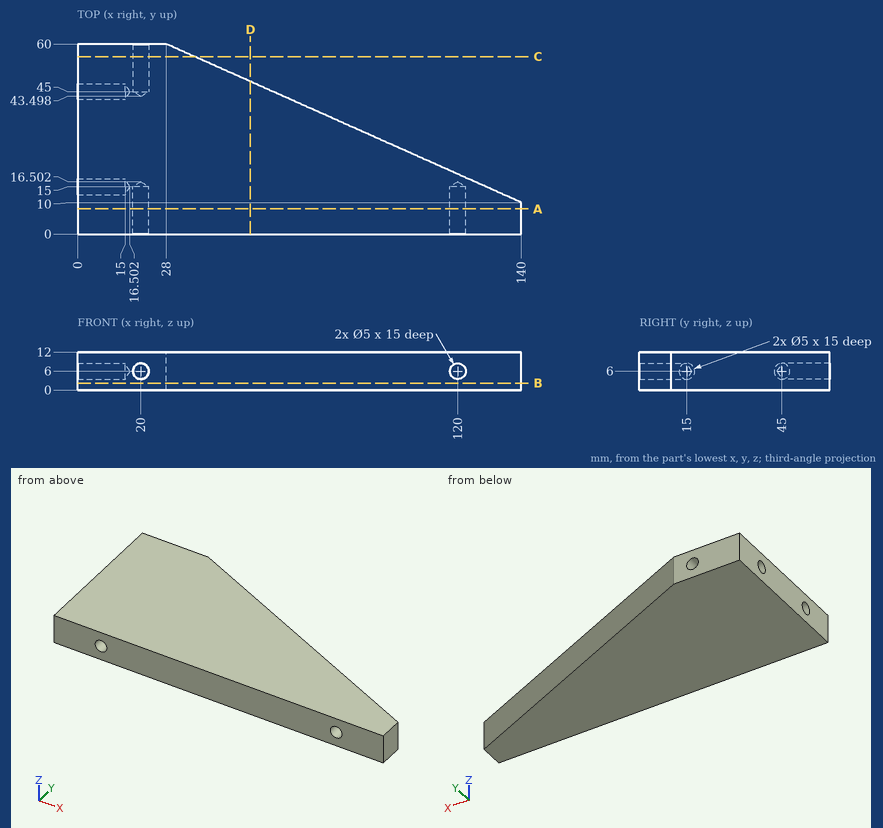
Part print with two shaded views. Sizes in mm from the minimum x, y, z corner. Round coordinates to 2 decimals unless told otherwise and drop trailing zeros. Order: outer loops, then holes, each group sorted by start corner. A loop starts at its lowest first (then second) coordinate and runs counter-clockwise, first axis right, second up. Notation, with made-up numbers: (14.25, -21.5) - (57.25, -21.5) arc R19 ccw to (57.25, -6.5) - close; hole circle Ø10 at (16, -27.5). An arc over 180 degrees is marked (long way). Answer in a Markdown table with one row per item. Add a question column.
(1) Band-saw the part on A-A on y = 8. List the corners of the cut face in (x, z).
(2) Band-saw the part on C-C on y = 56. List the corners of the cut face in (x, z).
(3) Band-saw the part on B-B on z = 2.25. List the corners of the cut face in (x, y).
(4) Probe L1, parallel to Y at x = 3.75, z = 6; L2, parallel to Z at x = 120, y = 8.25; L3, parallel to Y at x = 125.5, z = 11.5. List the from-to ranges inside material, lowest first. Write a range as [from, to].
(5) Band-saw the part on D-D on x = 54.5. List the corners of the cut face in (y, z).
(6) Drop flat-ended pins along their axis: pin 1 Ø3 at (x, z) = (20, 6) entering from +Y; pin 2 Ø5 at (x, z) = (122, 9) entering from +Y; pin 3 Ø4 at (y, z) = (45, 6) entering from +X. Give the stop position or say it passes through.
Data:
| question | item | result |
|---|---|---|
| 1 | outline | (0, 0) - (140, 0) - (140, 12) - (0, 12) - close; hole circle Ø5 at (20, 6); hole circle Ø5 at (120, 6) |
| 2 | outline | (0, 0) - (36.96, 0) - (36.96, 12) - (0, 12) - close; hole circle Ø5 at (20, 6) |
| 3 | outline | (0, 0) - (140, 0) - (140, 10) - (28, 60) - (0, 60) - close |
| 4 | L1 | y = [0, 12.5], [17.5, 42.5], [47.5, 60] |
| 4 | L2 | z = [0, 3.5], [8.5, 12] |
| 4 | L3 | y = [0, 16.47] |
| 5 | outline | (0, 0) - (48.17, 0) - (48.17, 12) - (0, 12) - close |
| 6 | pin 1 | stops at y = 44.4 |
| 6 | pin 2 | stops at y = 19.15 |
| 6 | pin 3 | stops at x = 66.08 |
